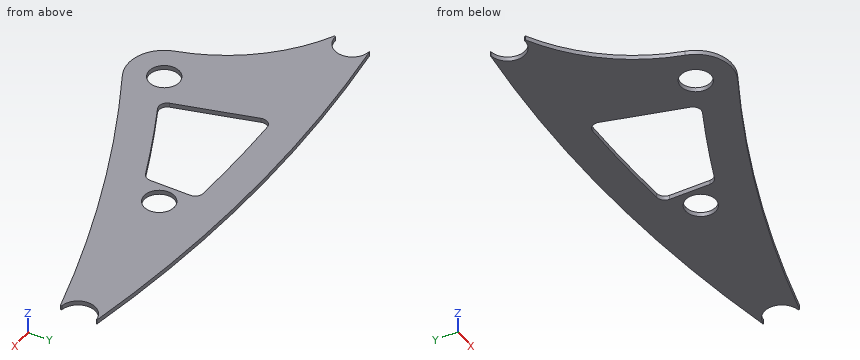
from build123d import *

# Parameters (mm, degrees)
SKETCH1_R           = 55
BOSS_EXTRUDE1_DEPTH = 16


with BuildPart() as part:
    # Sketch1 → Boss-Extrude1 (new body)
    with BuildSketch(Plane.XY):
        with BuildLine():
            Line((-441.486560332, 352.773302295), (-441.077967536, 357.443539322))
            ThreePointArc((-441.077967536, 357.443539322), (-371.743539322, 415.622032464), (-429.922032464, 484.956460678))
            Line((-429.922032464, 484.956460678), (-429.79492965, 486.409252487))
            ThreePointArc((-429.79492965, 486.409252487), (357.533978136, 521.031079354), (1140.522963582, 431.511647932))
            Line((1140.522963582, 431.511647932), (1140.708792797, 429.387610285))
            ThreePointArc((1140.708792797, 429.387610285), (1080.543840624, 367.868475852), (1135.99378326, 302.067797793))
            Line((1135.99378326, 302.067797793), (1136.4, 297.424719211))
            ThreePointArc((1136.4, 297.424719211), (586.381263284, 122.220397305), (60.221638572, -115.21004404))
            ThreePointArc((60.221638572, -115.21004404), (-51.454770489, -119.38344355), (-125.106294133, -35.332919047))
            ThreePointArc((-125.106294133, -35.332919047), (-243.082301892, 191.502339862), (-441.486560332, 352.773302295))
        make_face()
        Circle(SKETCH1_R, mode=Mode.SUBTRACT)
        with Locations((538, 300)):
            Circle(SKETCH1_R, mode=Mode.SUBTRACT)
        with BuildLine():
            Line((463, 367.628013441), (463, 222.86357491))
            ThreePointArc((463, 222.86357491), (457.896084334, 206.124847813), (444.32100101, 195.08165748))
            ThreePointArc((444.32100101, 195.08165748), (294.287770433, 131.138912095), (146.367210305, 62.450100371))
            ThreePointArc((146.367210305, 62.450100371), (121.015152193, 62.085681339), (104.438295549, 81.270766055))
            Line((104.438295549, 81.270766055), (24.221447422, 364.163456776))
            ThreePointArc((24.221447422, 364.163456776), (28.91122692, 390.115501396), (52.280902613, 402.336831507))
            ThreePointArc((52.280902613, 402.336831507), (243.460652484, 403.707205867), (434.547363171, 397.588081319))
            ThreePointArc((434.547363171, 397.588081319), (454.753400827, 388.286898998), (463, 367.628013441))
        make_face(mode=Mode.SUBTRACT)
    extrude(amount=BOSS_EXTRUDE1_DEPTH)


solid = part.part
Here's how the part is built. I have some questions about the finished solid (model axes, mm). Round coordinates to 2 decimals unless told otherwise and drop trailing zeros. Write each loop counter-clockwise with the first axis right and the second up, starting at its lowest first coordinate (ties: lowest second). Pieces come first, ordered by that corner, then holes.
1. Suppose I cut it at B-B (y = 0). List the corners of the cut face in (x, z) for me, and give its area (3 significant figures).
2. Will these pins go through, and if not, where does the flat tip stop? pin 1 Ø1.5 at (x, z) = (280.5, 4) entering from -Y; pin 2 Ø2 at (y, z) = (397.5, 9) entering from -X; pin 3 Ø5 at (y, z) = (184, 7.5) entering from -X.
3. Suppose I cut it at C-C (x = 538). List the corners of the cut face in (y, z) for me.
4. I need wall thicknesses on L1, parallel to X at y = 334, z = 8; L2, parallel to Y at x = 538, z = 10.75; L3, parallel to Y at x = 268, z = 7.5. Which ranges of each line are inside material? Lowest first, please.
5. Suppose I cut it at D-D (x = 839.5). List the corners of the cut face in (y, z) for me.
6. Suppose I cut it at A-A (z = 8.25). List the corners of the cut face in (x, y) for me.
Answer sheet:
1. outline: (-136.22, 0) - (-55, 0) - (-55, 16) - (-136.22, 16) - close; (55, 0) - (295.44, 0) - (295.44, 16) - (55, 16) - close
1. area: 5,150 mm2
2. pin 1: stops at y = -7.21
2. pin 2: stops at x = -376.46
2. pin 3: stops at x = -239.05
3. outline: (103.38, 0) - (245, 0) - (245, 16) - (103.38, 16) - close; (355, 0) - (511.45, 0) - (511.45, 16) - (355, 16) - close
4. L1: x = -407.83 to 32.77, 463 to 494.77, 581.23 to 1088.79
4. L2: y = 103.38 to 245, 355 to 511.45
4. L3: y = -12.66 to 119.35, 403.34 to 523.36
5. outline: (211.56, 0) - (480.78, 0) - (480.78, 16) - (211.56, 16) - close
6. outline: (-441.49, 352.77) arc R630 cw to (-125.11, -35.33) arc R130 ccw to (60.22, -115.21) arc R5000 cw to (1136.4, 297.42) - (1135.99, 302.07) arc R64 cw to (1140.71, 429.39) - (1140.52, 431.51) arc R5000 ccw to (-429.79, 486.41) - (-429.92, 484.96) arc R64 cw to (-441.08, 357.44) - close; hole circle Ø110 at (0, 0); hole (24.22, 364.16) - (104.44, 81.27) arc R30 ccw to (146.37, 62.45) arc R5120 cw to (444.32, 195.08) arc R30 ccw to (463, 222.86) - (463, 367.63) arc R30 ccw to (434.55, 397.59) arc R4880 ccw to (52.28, 402.34) arc R30 ccw to start; hole circle Ø110 at (538, 300)
